Input: part model. Units: mm. Frame: model coordinates. A direction names the side the tool comes from. Coordinates: 2 decimals unless noted, no trailing zeros. Order: outer loops, then holes, each group sorted by start corner. A loop starts at its lowest first (then second) coordinate and runs counter-clockwise, first axis right, second up. Notation, with made-up numbers: (89, -23.5) -> (99, -23.5) arc R15 ccw to (99, 1.5) -> close; hole circle Ø7 at (-23.5, 33). An arc over 180 degrees is marked (long way). Write each question's results on one line, items separated by ' | '.
```python
from build123d import *

# Parameters (mm, degrees)
SKETCH_1_R          = 15.75
SKETCH_1_R_2        = 1.6
EXTRUDE_1_DEPTH     = 3
SKETCH_2_W          = 28.7
SKETCH_2_H          = 68.308962896
CUT_EXTRUDE_1_DEPTH = 93.750249245
FILLET_1_R          = 12
SKETCH_4_R          = 1.6
CUT_EXTRUDE_2_DEPTH = 93.750249245
SKETCH_5_R          = 4.5
SKETCH_5_R_2        = 1.6
EXTRUDE_2_DEPTH     = 3
FILLET_2_R          = 2


with BuildPart() as part:
    # 草图1 → 凸台-拉伸1 (new body)
    with BuildSketch(Plane(origin=(0, 0, 0), x_dir=(0, 0, -1), z_dir=(1, 0, 0))):
        with BuildLine():
            Line((18.093011091, 18.671983014), (24, 27.077468597))
            Line((24, 27.077468597), (22, 71.98094591))
            Line((22, 71.98094591), (22, 88.98094591))
            Line((22, 88.98094591), (-24.8, 88.98094591))
            Line((-24.8, 88.98094591), (-24.8, 70.98094591))
            Line((-24.8, 70.98094591), (-25.996262077, 0.440860573))
            ThreePointArc((-25.996262077, 0.440860573), (9.935230264, -24.026884933), (18.093011091, 18.671983014))
        make_face()
        Circle(SKETCH_1_R, mode=Mode.SUBTRACT)
        with Locations((14.000714267, 14.000714267)):
            Circle(SKETCH_1_R_2, mode=Mode.SUBTRACT)
        with Locations((14.000714267, -14.000714267)):
            Circle(SKETCH_1_R_2, mode=Mode.SUBTRACT)
        with Locations((-14.000714267, -14.000714267)):
            Circle(SKETCH_1_R_2, mode=Mode.SUBTRACT)
        with Locations((-14.000714267, 14.000714267)):
            Circle(SKETCH_1_R_2, mode=Mode.SUBTRACT)
        with Locations((-20.8, 84.98094591)):
            Circle(SKETCH_1_R_2, mode=Mode.SUBTRACT)
        with Locations((-20.8, 76.98094591)):
            Circle(SKETCH_1_R_2, mode=Mode.SUBTRACT)
        with Locations((18, 84.98094591)):
            Circle(SKETCH_1_R_2, mode=Mode.SUBTRACT)
        with Locations((18, 76.98094591)):
            Circle(SKETCH_1_R_2, mode=Mode.SUBTRACT)
    extrude(amount=EXTRUDE_1_DEPTH)

    # 草图2 → 切除-拉伸1 (cut, through all)
    with BuildSketch(Plane.ZY):
        with Locations((0.45, 54.826464462)):
            Rectangle(SKETCH_2_W, SKETCH_2_H)
    extrude(amount=-CUT_EXTRUDE_1_DEPTH, mode=Mode.SUBTRACT)

    # 圆角1
    fillet_1_edges = [part.edges().sort_by_distance(p)[0] for p in [
        (1.5, 20.671983014, -13.9),
        (1.5, 20.671983014, 14.8),
    ]]
    fillet(fillet_1_edges, radius=FILLET_1_R)

    # 草图4 → 切除-拉伸2 (cut, through all)
    with BuildSketch(Plane(origin=(3, 0, 0), x_dir=(0, 0, -1), z_dir=(1, 0, 0))):
        with Locations((-17, 44.000714267)):
            Circle(SKETCH_4_R)
        with Locations((17, 44.000714267)):
            Circle(SKETCH_4_R)
    extrude(amount=-CUT_EXTRUDE_2_DEPTH, mode=Mode.SUBTRACT)

    # 草图5 → 凸台-拉伸2 (add)
    # profile 1 of 3: a face of its own
    with BuildSketch(Plane(origin=(3, 0, 0), x_dir=(0, 0, -1), z_dir=(1, 0, 0))):
        with Locations((-17, 44.000714267)):
            Circle(SKETCH_5_R)
        with Locations((-17, 44.000714267)):
            Circle(SKETCH_5_R_2, mode=Mode.SUBTRACT)
    # profile 2 of 3: a face of its own
    with BuildSketch(Plane(origin=(3, 0, 0), x_dir=(0, 0, -1), z_dir=(1, 0, 0))):
        with Locations((17, 44.000714267)):
            Circle(SKETCH_5_R)
        with Locations((17, 44.000714267)):
            Circle(SKETCH_5_R_2, mode=Mode.SUBTRACT)
    # profile 3 of 3: a face of its own
    with BuildSketch(Plane(origin=(3, 0, 0), x_dir=(0, 0, -1), z_dir=(1, 0, 0))):
        with BuildLine():
            Line((-12.394227472, -35.784446941), (-23.70501151, -10.680469528))
            ThreePointArc((-23.70501151, -10.680469528), (-6.729295173, -25.114071484), (15.1889074, -21.10206369))
            Line((15.1889074, -21.10206369), (-7.158507619, -37.187353847))
            ThreePointArc((-7.158507619, -37.187353847), (-10.109034889, -37.72743182), (-12.394227472, -35.784446941))
        make_face()
        with Locations((-9.203168231, -34.346691428)):
            Circle(SKETCH_5_R_2, mode=Mode.SUBTRACT)
    extrude(amount=-EXTRUDE_2_DEPTH)

    # 圆角2
    fillet_2_edges = [part.edges().sort_by_distance(p)[0] for p in [
        (1.5, 47.926271553, 14.8),
        (1.5, 40.075156982, 14.8),
        (1.5, 70.98094591, 24.8),
        (1.5, 88.98094591, 24.8),
        (1.5, 88.98094591, -22),
        (1.5, 71.98094591, -22),
        (1.5, 27.077468597, -24),
        (1.5, 40.738812981, -13.9),
        (1.5, 18.671983014, -18.093011091),
        (1.5, 47.262615554, -13.9),
        (1.5, 88.98094591, -13.9),
        (1.5, 88.98094591, 14.8),
    ]]
    fillet(fillet_2_edges, radius=FILLET_2_R)


solid = part.part
```
(1) Cut plane A-A, the plane z = 4. Return loops of the section in (x, y), plus the area to 3 significant figures.
Return value:
outline: (0, -34.91) -> (3, -34.91) -> (3, -15.23) -> (0, -15.23) -> close; (0, 15.23) -> (3, 15.23) -> (3, 20.73) -> (0, 20.73) -> close | area: 75.5 mm2
(2) Mould query, pull axis Z, two halves, no side actions, for faces 1 (the face through (0, 12, 12)), 2 (the face through (1, 20.672, 0)), 3 (the face through (1, 79, 24.8)). Classes: +Z half, -Z half, draft (parallel to the pull), parting line (faces both ways), or undercut.
Return value:
face 1: draft | face 2: undercut | face 3: +Z half
(3) Pin query (flat end, axial travel): P1, Ø4, axis at y = 44, z = -17, coming from the -X side; P2, Ø3, axis at y = 14, z = 14, coming from the +X side; P3, Ø1.5, axis at x = 1, y = 18, coming from the +Z side; P4, Ø0.9, axis at x = 2, y = 69.5, coming from the +Z side. Return the tip coordinate at first contact, or that it passes through.
Return value:
P1: x = 0 | P2: through | P3: z = 25.71 | P4: z = 24.83
(4) Cut plane D-D, the plane x = 1.25. Count the separate pieces of the cut face and the enclosed holes in it, plus the area to 3 significant figures.
Return value:
separate pieces: 1 | enclosed holes: 12 | area: 2,810 mm2
(5) Cut plane B-B, the plane y = 9. Return loops of the section in (x, z), plus the area to 3 significant figures.
Return value:
outline: (0, -24.39) -> (3, -24.39) -> (3, -12.93) -> (0, -12.93) -> close; (0, 12.93) -> (3, 12.93) -> (3, 25.85) -> (0, 25.85) -> close | area: 73.2 mm2
(6) Cut plane C-C, the plane z = 20.8. Return loops of the section in (x, y).
Return value:
outline: (0, -17.13) -> (3, -17.13) -> (3, 75.38) -> (0, 75.38) -> close; (0, 78.58) -> (3, 78.58) -> (3, 83.38) -> (0, 83.38) -> close; (0, 86.58) -> (3, 86.58) -> (3, 88.98) -> (0, 88.98) -> close
(7) Reachability of faces 4 (the face through (1.48, 49.56, -23)), 5 (the face through (1.5, 44, -12.5)) from +Z, -Z, +X, -X, +Y, -Y: full face, straight path, thin tool, end or side. Return the list, or none.
Return value:
face 4: -Z, +X, -X, +Y | face 5: +X, -X
(8) Line query: line 1 along Y through (x, z) = (1.35, -18); line 2 along Z through (x, y) = (0.9, 44); line 3 along Y through (x, z) = (1.95, -17). Output: solid intervals per line, ascending. Write a range as from..to.
Return value:
line 1: -18.76..42.75, 45.25..75.38, 78.58..83.38, 86.58..88.98 | line 2: -23.25..-18.6, -15.4..-12.5, 12.5..15.4, 18.6..25.26 | line 3: -19.67..42.4, 45.6..75.73, 78.23..83.73, 86.23..88.98
